from build123d import *


with BuildPart() as part:
    # Sketch1 → Revolve1 (revolve)
    with BuildSketch(Plane.XY, mode=Mode.PRIVATE) as revolve1_sk:
        Polygon((25.5, 60), (25.5, 20), (12.5, 20), (12.5, 0), (50, 0), (50, 20), (30.5, 20), (30.5, 60), align=None)
    revolve(revolve1_sk.sketch.rotate(Axis((0, 0, 0), (0, 1, 0)), 90), axis=Axis((0, 0, 0), (0, 1, 0)))


solid = part.part
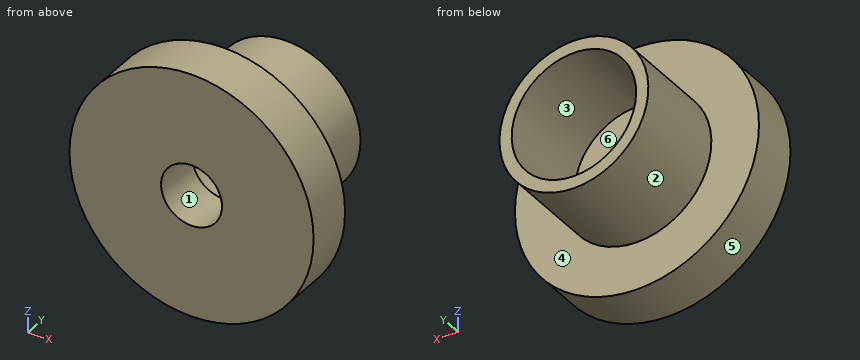
Work out the finished part from the listing and answer in its coordinate system (mm). Face numbers are marked on the shaded views. A direction names the side the tool comes from. Coordinates: 2 decimals unless noted, no trailing zeros. Write each loop counter-clockwise with the first axis right and the second up, starting at its lowest first coordinate (ties: lowest second). Pieces come first, ordered by that corner, then holes. Notation, with made-up numbers: (16, 50.25) - (74, 50.25) arc R28 cw to (74, 78.25) - close; hole circle Ø4 at (11, 88.5). An arc over 180 degrees is marked (long way). One line per question, with ' | ' between items.
1) Flat-ended cylindrical pins translate along their axes: P1, Ø1, axis at y = 39, z = -4.5, coming from the -X side; P2, Ø12, axis at y = 46.5, z = 2, coming from the +X side; P3, Ø4, axis at x = 18, y = 44, coming from the +Z side. Find the tip coordinate at first contact, or state that the pin passes through.
Checks:
P1: x = -30.24 | P2: x = 30.5 | P3: z = 25.97
2) Find section B-B, the plane x = 0. Determine the outline of the cut face in (y, z).
Checks:
outline: (0, -50) - (20, -50) - (20, -30.5) - (60, -30.5) - (60, -25.5) - (20, -25.5) - (20, -12.5) - (0, -12.5) - close; (0, 12.5) - (20, 12.5) - (20, 25.5) - (60, 25.5) - (60, 30.5) - (20, 30.5) - (20, 50) - (0, 50) - close
3) Find section D-D, the plane x = 14.5. Determine the outline of the cut face in (y, z).
Checks:
outline: (0, -47.85) - (20, -47.85) - (20, -26.83) - (60, -26.83) - (60, -20.98) - (20, -20.98) - (20, 20.98) - (60, 20.98) - (60, 26.83) - (20, 26.83) - (20, 47.85) - (0, 47.85) - close
4) The mould has two halves that part along Z. Classify the marked faces 3, 4, 5 and 6: +Z half, -Z half, draft (parallel to the pull), parting line (faces both ways), or undercut.
Checks:
face 3: undercut | face 4: draft | face 5: parting line | face 6: undercut
5) For the marked faces 1 and 2, determine the directions among +Z, -Z, +X, -X, +Y, -Y from which every point of the face is accessible in a straight line to the end or side of a thin tool.
Checks:
face 1: +Y, -Y | face 2: +Y
6) Consider probe 1 along X at (y, z) = (49.5, 0); probe 2 along X at (y, z) = (9, 0); probe 3 along Y at (x, z) = (15.5, 19). Determine where each line is inside the solid, lowest interval first. Write a range as [from, to].
Checks:
probe 1: [-30.5, -25.5], [25.5, 30.5] | probe 2: [-50, -12.5], [12.5, 50] | probe 3: [0, 20]
7) Find section C-C, the plane y = 5. Determine the outline of the cut face in (x, z), and give its area (3 significant figures).
Checks:
outline: circle Ø100 at (0, 0); hole circle Ø25 at (0, 0) | area: 7,360 mm2
8) Find section A-A, the plane z = 0. Determine the outline of the cut face in (x, y).
Checks:
outline: (-50, 0) - (-12.5, 0) - (-12.5, 20) - (-25.5, 20) - (-25.5, 60) - (-30.5, 60) - (-30.5, 20) - (-50, 20) - close; (12.5, 0) - (50, 0) - (50, 20) - (30.5, 20) - (30.5, 60) - (25.5, 60) - (25.5, 20) - (12.5, 20) - close
